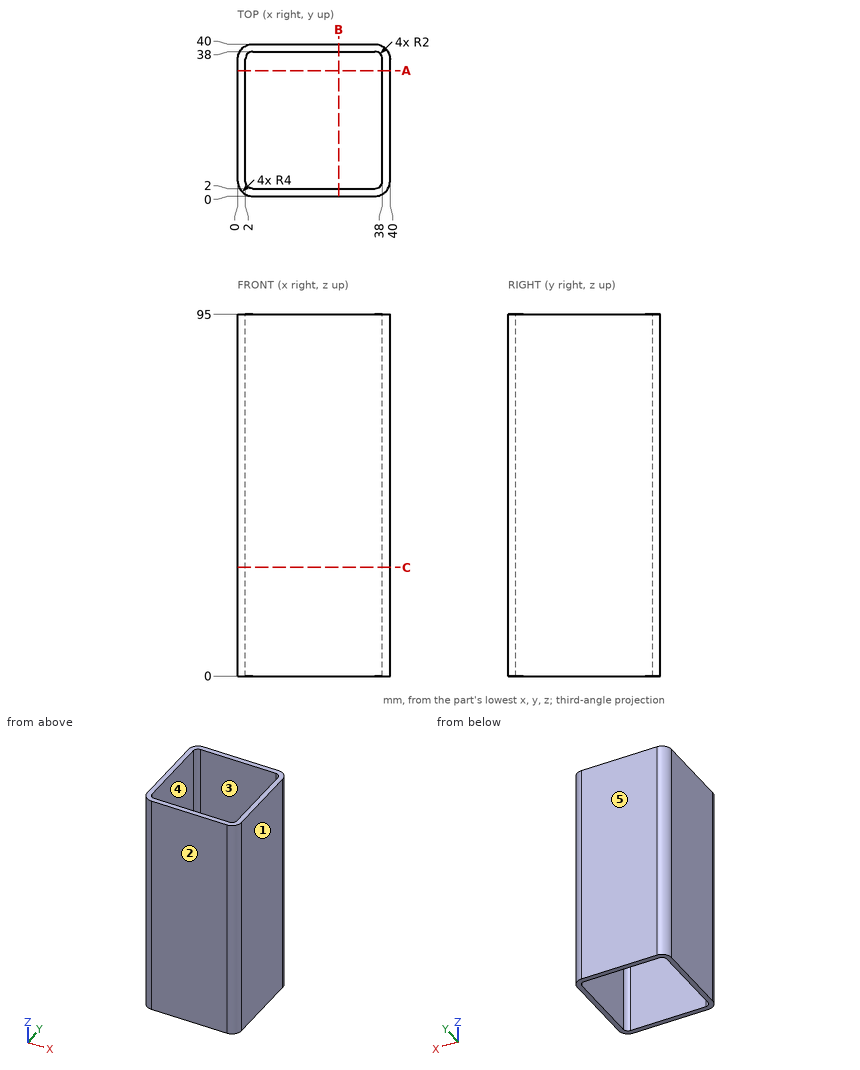
Job drawing, mm, ordinate dimensions from the low corner. One solid piece. A direction names the side the tool comes from. Give positions to 0.01 mm unless a question says otherwise; leave off trailing zeros. Order: outer loops, then holes, each group sorted by start corner. A loop starts at its lowest first (then second) coordinate and runs counter-clockwise, first axis right, second up. Notation, with made-up numbers: (72, 72) -> (108, 72) arc R11 cw to (108, 88) -> close; hole circle Ø5 at (-30.5, 36). An arc over 180 degrees is marked (long way). Return JSON: item names as keys, results as strings.
Q1. Saw through at C-C (z = 28.5). Write the cut outline in (x, y).
Working result:
{"outline": "(0, 4) arc R4 ccw to (4, 0) -> (36, 0) arc R4 ccw to (40, 4) -> (40, 36) arc R4 ccw to (36, 40) -> (4, 40) arc R4 ccw to (0, 36) -> close; hole (2, 4) arc R2 ccw to (4, 2) -> (36, 2) arc R2 ccw to (38, 4) -> (38, 36) arc R2 ccw to (36, 38) -> (4, 38) arc R2 ccw to (2, 36) -> close"}
Q2. Which spindle directions (+Z, -Z, +X, -X, +Y, -Y) get a long thin tool onto all of the face, cutting with end or side? Do the marked faces 4 and 5. Say none if no direction does.
Working result:
{"face 4": "+Z, -Z", "face 5": "+Z, -Z, +X, -X, +Y"}
Q3. Mould opens along X. For the marked faces 1, 2 and 3 say: pulls with the +X half, pulls with the -X half, needs draft (parallel to the pull), parting line crosses it, or undercut.
Working result:
{"face 1": "pulls with the +X half", "face 2": "needs draft", "face 3": "undercut"}
Q4. Flat gauge pin, fed straight in: pin 1 (5 mm diameter, centred on x = 34, y = 13.5, fed in from +Z). Where does the tip first touch, or does it go through?
Working result:
{"pin 1": "through"}
Q5. Saw through at A-A (y = 33). Write the cut outline in (x, z), then the cut area to 3 significant figures.
Working result:
{"outline": "(0, 0) -> (2, 0) -> (2, 95) -> (0, 95) -> close; (38, 0) -> (40, 0) -> (40, 95) -> (38, 95) -> close", "area": "380 mm²"}
Q6. Drill centre lines: line 1 (Y direction, x = 13, z = 91); line 2 (X direction, y = 37, z = 6.5). Where is each one in solid material? Low to high.
Working result:
{"line 1": "0 to 2, 38 to 40", "line 2": "0.13 to 2.27, 37.73 to 39.87"}
